Check sheet for the modelled part. Datum: model origin and axes. Units: mm. Face numbers are marked on the shaded views. Coordinates: 2 decimals unless noted, no trailing zeros. Loops run counter-clockwise (first coordinate to the right, second up) from the corner with the lowest first, then second, coordinate; pieces in that order, holes last. Notation, with made-up numbers: M -21,15.25 L 29,15.25 A16 cw 29,23.25 Z; hole C -25.75,34 d4. An arc over 180 degrees is marked long. Answer in a Markdown table with one row per item. Add a question column.
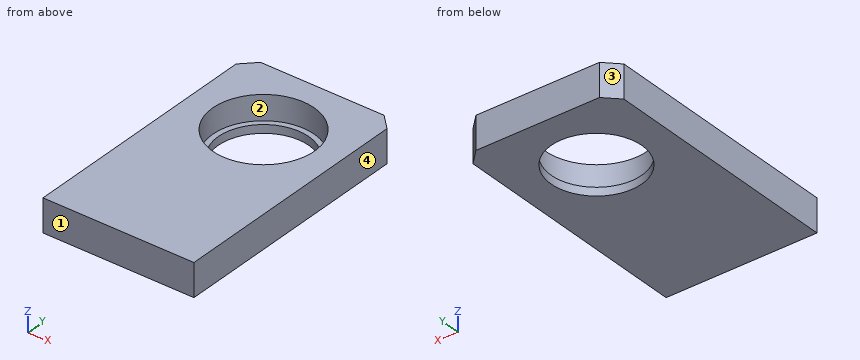
```python
from build123d import *

# Parameters (mm, degrees)
SKETCH_1_W          = 55
SKETCH_1_H          = 94.5
EXTRUDE_1_DEPTH     = 12
CUT_EXTRUDE_4_REACH = 57.972
SKETCH_5_R          = 18.5
CHAMFER_1_SIZE      = 5
SKETCH_6_R          = 18.5
SKETCH_6_R_2        = 16.5
EXTRUDE_2_DEPTH     = 3


with BuildPart() as part:
    # 草图1 → 凸台-拉伸1 (new body)
    with BuildSketch(Plane.XY):
        Rectangle(SKETCH_1_W, SKETCH_1_H)
    extrude(amount=EXTRUDE_1_DEPTH)

    # 草图5 → 切除-拉伸4 (cut, up to next)
    with BuildSketch(Plane(origin=(0, 0, 0), x_dir=(-1, 0, 0), z_dir=(0, 0, -1)), mode=Mode.PRIVATE) as cut_extrude_4_sk1:
        with Locations((0, 20)):
            Circle(SKETCH_5_R)
    cut_extrude_4_tool1 = extrude(cut_extrude_4_sk1.sketch, amount=-CUT_EXTRUDE_4_REACH, mode=Mode.PRIVATE) & part.part
    add(cut_extrude_4_tool1.solids().sort_by_distance((0, 20, 0))[0], mode=Mode.SUBTRACT)

    # 倒角1
    chamfer_1_edges = [part.edges().sort_by_distance(p)[0] for p in [
        (-27.5, 47.25, 6),
        (27.5, 47.25, 6),
    ]]
    chamfer(chamfer_1_edges, length=CHAMFER_1_SIZE)

    # 草图6 → 凸台-拉伸2 (add)
    with BuildSketch(Plane(origin=(0, 0, 0), x_dir=(-1, 0, 0), z_dir=(0, 0, -1))):
        with Locations((0, 20)):
            Circle(SKETCH_6_R)
        with Locations((0, 20)):
            Circle(SKETCH_6_R_2, mode=Mode.SUBTRACT)
    extrude(amount=-EXTRUDE_2_DEPTH)


solid = part.part
```
Q1. Cross-section at A-A (x = 0). Record the cut outline in (y, z).
Q2. Cross-section at C-C (y = 20). Record the cut outline in (x, z).
Q3. Cross-section at B-B (z = 5.5). Record the cut outline in (x, y).
Q4. Mould release check, pull along Y, two halves, no side actions. Record for the marked faces 1, 2, 3 and 4: released by +Y, released by -Y, zero draft, split by the parting line, or undercut.
Q5. Go/stop test with flat-tipped pins: pin 1 (1 mm diameter, centred on x = 6, y = -29.5, fed in from -Z); pin 2 (18.5 mm diameter, centred on x = 1.5, y = 12, fed in from +Z). Record where each tip stops, or that it passes through.
Q6. Thickness scan on L1, parallel to Y at x = 0, z = 6.5; L2, parallel to Y at x = -17, z = 4.5; L3, parallel to X at y = 13, z = 2.5. Record the ranges inside material, lowest first.
Answer key:
| question | item | result |
|---|---|---|
| 1 | outline | M -47.25,0 L 3.5,0 L 3.5,3 L 1.5,3 L 1.5,12 L -47.25,12 Z; M 36.5,0 L 47.25,0 L 47.25,12 L 38.5,12 L 38.5,3 L 36.5,3 Z |
| 2 | outline | M -27.5,0 L -16.5,0 L -16.5,3 L -18.5,3 L -18.5,12 L -27.5,12 Z; M 16.5,0 L 27.5,0 L 27.5,12 L 18.5,12 L 18.5,3 L 16.5,3 Z |
| 3 | outline | M -27.5,-47.25 L 27.5,-47.25 L 27.5,42.25 L 22.5,47.25 L -22.5,47.25 L -27.5,42.25 Z; hole C 0,20 d37 |
| 4 | face 1 | released by -Y |
| 4 | face 2 | undercut |
| 4 | face 3 | released by +Y |
| 4 | face 4 | zero draft |
| 5 | pin 1 | z = 0 |
| 5 | pin 2 | z = 3 |
| 6 | L1 | -47.25 to 1.5, 38.5 to 47.25 |
| 6 | L2 | -47.25 to 12.7, 27.3 to 47.25 |
| 6 | L3 | -27.5 to -14.94, 14.94 to 27.5 |
